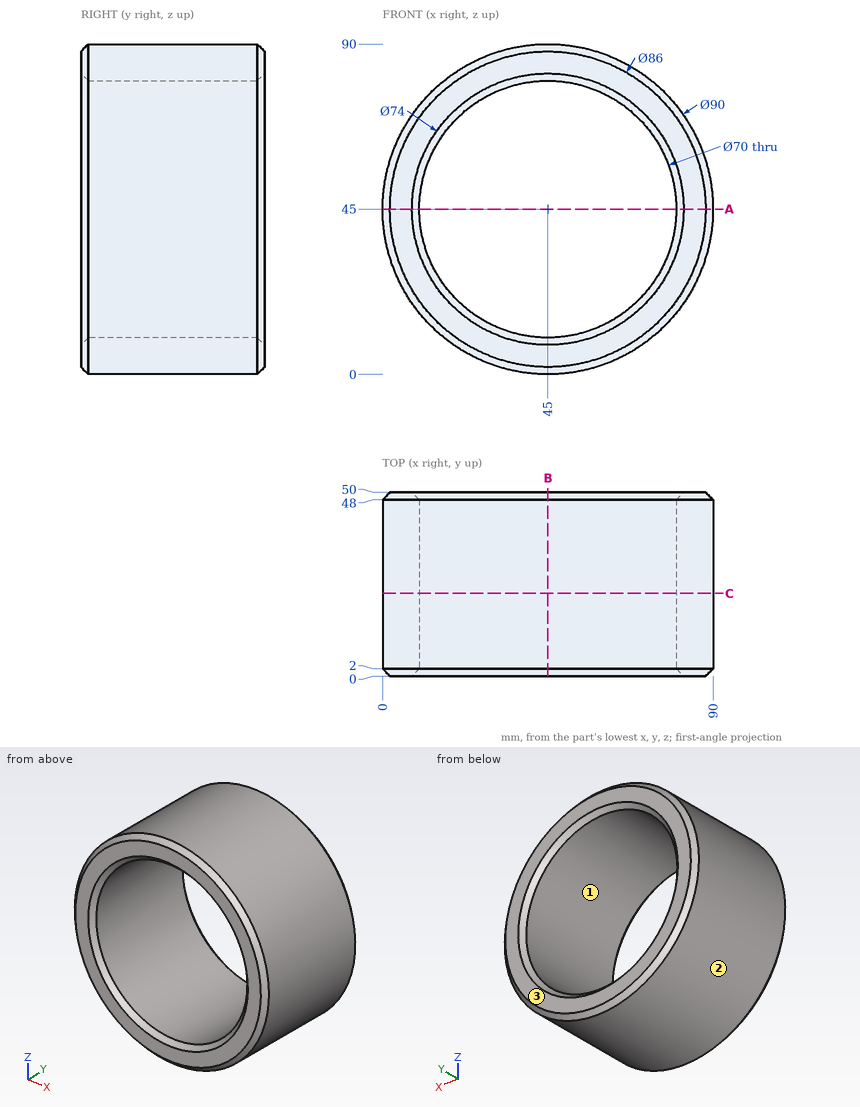
Print and shaded views of the part. All mm, measured from the part's lowest x, y and z. Round coordinates to 2 decimals unless told otherwise and drop trailing zeros. Write each loop counter-clockwise with the first axis right and the second up, starting at its lowest first coordinate (ties: lowest second). Pieces come first, ordered by that corner, then holes. Notation, with made-up numbers: M 47.25,-40 L 90.25,-40 A16 ccw 90.25,-17 Z; hole C 86.25,31.25 d11. An arc over 180 degrees is marked long. Use a Markdown table: item, result. Add a question column.
1. Slice it at C-C on y = 22.5. Give the cut face in (x, z), then the cut area to 3 significant figures.
2. Flat gauge pins, fed straight in: P1, Ø6, axis at y = 34.5, z = 23, coming from the +X side; P2, Ø5, axis at y = 10, z = 12, coming from the -X side; P3, Ø3, axis at y = 44, z = 43.5, coming from the -X side. Where does each tip first touch, or does it go through?
3. Drill centre lines: probe 1 along X at (y, z) = (28, 45); probe 2 along Z at (x, y) = (36, 12); probe 3 along X at (y, z) = (25.5, 65). Where is each one in solid material? Low to high.
4. Slice it at B-B on x = 45. Give the cut face in (y, z).
5. Slice it at A-A on z = 45. Give the cut face in (x, y), then the cut area to 3 significant figures.
6. Pull direction Z, two halves, no side cores. Call the marked faces 1, 2 and 3: released by +Z, released by -Z, zero draft, split by the parting line, or undercut.
Reply:
| question | item | result |
|---|---|---|
| 1 | outline | C 45,45 d90; hole C 45,45 d70 |
| 1 | area | 2,510 mm^2 |
| 2 | P1 | stops at x = 85.79 |
| 2 | P2 | stops at x = 11.91 |
| 2 | P3 | stops at x = 0 |
| 3 | probe 1 | x = 0 to 10, 80 to 90 |
| 3 | probe 2 | z = 0.91 to 11.18, 78.82 to 89.09 |
| 3 | probe 3 | x = 4.69 to 16.28, 73.72 to 85.31 |
| 4 | outline | M 0,2 L 2,0 L 48,0 L 50,2 L 50,8 L 48,10 L 2,10 L 0,8 Z; M 0,82 L 2,80 L 48,80 L 50,82 L 50,88 L 48,90 L 2,90 L 0,88 Z |
| 5 | outline | M 0,2 L 2,0 L 8,0 L 10,2 L 10,48 L 8,50 L 2,50 L 0,48 Z; M 80,2 L 82,0 L 88,0 L 90,2 L 90,48 L 88,50 L 82,50 L 80,48 Z |
| 5 | area | 984 mm^2 |
| 6 | face 1 | undercut |
| 6 | face 2 | split by the parting line |
| 6 | face 3 | zero draft |
